Design review of the part built by this model. Coordinates are the model's own, in mm. Coordinates: 2 decimals unless noted, no trailing zeros. Write each loop counter-clockwise with the first axis right and the second up, starting at its lowest first coordinate (ties: lowest second). Pieces come first, ordered by that corner, then holes.
Q1. For L1, parallel to Y at x = 0, z = 1.8; L2, parallel to Y at x = 2.25, z = 1.9; L3, parallel to Y at x = -12.75, z = 2, list the stretches that pass through material, from the lowest coordinate up.
Q2. Take a section at D-D, the plane x = 13.25. Write out the cut boundary in (y, z).
Q3. Take a section at B-B, the plane x = 0. Write out the cut boundary in (y, z).
Q4. Take a section at C-C, the plane z = 1.1. Write out the cut boundary in (x, y).
Q5. For pin 1 Ø1 at (x, y) = (6, -4) entering from -Z, flat-tipped, find the tip position at first contact; note if it passes through.
Q6. Take a section at A-A, the plane y = -20. Write out the cut boundary in (x, z).
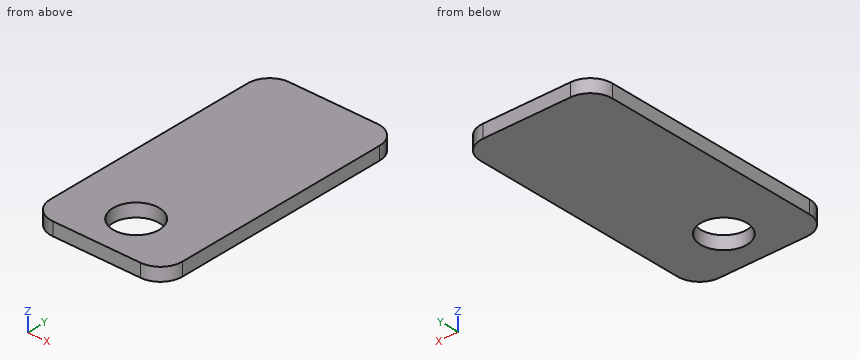
from build123d import *

# Parameters (mm, degrees)
SKETCH1_R           = 5.25
BOSS_EXTRUDE1_DEPTH = 3


with BuildPart() as part:
    # Sketch1 → Boss-Extrude1 (new body)
    with BuildSketch(Plane.XY):
        with BuildLine():
            Line((-10, 30), (10, 30))
            ThreePointArc((10, 30), (13.535533906, 28.535533906), (15, 25))
            Line((15, 25), (15, -25))
            ThreePointArc((15, -25), (13.535533906, -28.535533906), (10, -30))
            Line((10, -30), (-10, -30))
            ThreePointArc((-10, -30), (-13.535533906, -28.535533906), (-15, -25))
            Line((-15, -25), (-15, 25))
            ThreePointArc((-15, 25), (-13.535533906, 28.535533906), (-10, 30))
        make_face()
        with Locations((0, -20)):
            Circle(SKETCH1_R, mode=Mode.SUBTRACT)
    extrude(amount=BOSS_EXTRUDE1_DEPTH)


solid = part.part
Responses:
1. L1: y = -30 to -25.25, -14.75 to 30
1. L2: y = -30 to -24.74, -15.26 to 30
1. L3: y = -29.18 to 29.18
2. outline: (-28.8, 0) - (28.8, 0) - (28.8, 3) - (-28.8, 3) - close
3. outline: (-30, 0) - (-25.25, 0) - (-25.25, 3) - (-30, 3) - close; (-14.75, 0) - (30, 0) - (30, 3) - (-14.75, 3) - close
4. outline: (-15, -25) arc R5 ccw to (-10, -30) - (10, -30) arc R5 ccw to (15, -25) - (15, 25) arc R5 ccw to (10, 30) - (-10, 30) arc R5 ccw to (-15, 25) - close; hole circle Ø10.5 at (0, -20)
5. pin 1: stops at z = 0
6. outline: (-15, 0) - (-5.25, 0) - (-5.25, 3) - (-15, 3) - close; (5.25, 0) - (15, 0) - (15, 3) - (5.25, 3) - close
